The model under review builds one solid part; all positions refer to its coordinate system, in mm. A direction names the side the tool comes from. Give positions to 0.01 mm unless a question says otherwise; leave off trailing zeros. Write each loop counter-clockwise with the first axis right and the second up, starting at its lowest first coordinate (ties: lowest second). Pieces come first, ordered by that corner, then holes. Notation, with made-up numbers: (52.5, -39) - (93.5, -39) arc R21 ccw to (93.5, -8) - close; hole circle Ø4 at (36.25, 31). An arc over 180 degrees is marked (long way). Write item = value, one per line.
```python
from build123d import *

# Parameters (mm, degrees)
SKETCH_1_R               = 5
EXTRUDE_1_DEPTH          = 10
SKETCH_2_R               = 2
EXTRUDE_2_DEPTH          = 6
SKETCH_3_W               = 0.3
SKETCH_3_H               = 0.5
HOLE_WIZARD_M4_1_D       = 3.3
HOLE_WIZARD_M4_1_DEPTH   = 10.1
HOLE_WIZARD_M4_1_TIP     = 0.991420021
CHAMFER_1_SIZE           = 0.5
CUT_EXTRUDE_1_DEPTH      = 18.492855685
CUT_EXTRUDE_1_DEPTH_BACK = 18.492855685
SKETCH_6_R               = 2.25


with BuildPart() as part:
    # 草图1 → 凸台-拉伸1 (new, symmetric)
    with BuildSketch(Plane(origin=(0, 0, 0), x_dir=(1, 0, 0), z_dir=(0, 1, 0))):
        with Locations(Location((0, 0, 0), (0, 0, 270))):
            Circle(SKETCH_1_R)
    extrude(amount=EXTRUDE_1_DEPTH, both=True)

    # 草图2 → 凸台-拉伸2 (add)
    with BuildSketch(Plane.XZ.offset(10)):
        with Locations(Location((0, 0, 0), (0, 0, 90))):
            Circle(SKETCH_2_R)
    extrude(amount=EXTRUDE_2_DEPTH)

    # 草图3 → 切除-旋转1 (revolve, cut)
    with BuildSketch(Plane.XY, mode=Mode.PRIVATE) as cut_revolve_1_sk:
        with Locations((1.85, -10.25)):
            Rectangle(SKETCH_3_W, SKETCH_3_H)
    revolve(cut_revolve_1_sk.sketch.rotate(Axis((0, 0, 0), (0, -1, 0)), 90), axis=Axis((0, 0, 0), (0, -1, 0)), mode=Mode.SUBTRACT)

    # M4 螺纹孔1
    with Locations(Plane(origin=(0, 10, 0), x_dir=(1, 0, 0), z_dir=(0, 1, 0))):
        with Locations((0, 0)):
            Hole(HOLE_WIZARD_M4_1_D / 2, depth=HOLE_WIZARD_M4_1_DEPTH)
            with Locations((0, 0, -(HOLE_WIZARD_M4_1_DEPTH + HOLE_WIZARD_M4_1_TIP / 2))):  # 118° drill point
                Cone(0, HOLE_WIZARD_M4_1_D / 2, HOLE_WIZARD_M4_1_TIP, mode=Mode.SUBTRACT)

    # 倒角1
    chamfer_1_edges = [part.edges().sort_by_distance(p)[0] for p in [
        (0, -10, -5),
        (0, 10, -5),
    ]]
    chamfer(chamfer_1_edges, length=CHAMFER_1_SIZE)

    # 草图6 → 切除-拉伸1 (cut, two sides: drawn at the far end of the back side and taken through both)
    with BuildSketch(Plane(origin=(0, 0, 0), x_dir=(0, 0, -1), z_dir=(1, 0, 0)).offset(-CUT_EXTRUDE_1_DEPTH_BACK)):
        Circle(SKETCH_6_R)
    extrude(amount=CUT_EXTRUDE_1_DEPTH + CUT_EXTRUDE_1_DEPTH_BACK, mode=Mode.SUBTRACT)


solid = part.part
```
1. Machinability: for faces 4 (the flat face through (-2, 10, 0)), 5 (the cylindrical face through (1.66, -10.25, -0.37)), 6 (the cylindrical face through (2, -13, 0)), which of the approach directions +Z, -Z, +X, -X, +Y, -Y give a long, thin tool a straight path to every point of the face, cutting with its end or side? Answer none if there is none.
Findings below:
face_4 = +Z, -Z, +X, -X, +Y
face_5 = none
face_6 = -Y
2. For line 1 (Y direction, x = 3.25, z = 0); line 2 (Z direction, x = 0.25, y = 0); line 3 (Y direction, x = -1.75, z = 0.25), list the stretches that pass through material, from the lowest coordinate up. Write a range as from..to.
Findings below:
line_1 = -10..-2.25, 2.25..10
line_2 = -4.99..-2.25, 2.25..4.99
line_3 = -16..-10.5, -10..-2.24, 2.24..10
3. Insertion check: P1, Ø6, axis at y = 0, z = 0, coming from the +X side; P2, Ø3, axis at y = -8.5, z = -2, coming from the -X side; P3, Ø1, axis at x = 1, z = -0.5, coming from the +Y side; P4, Ø4, axis at x = 3.5, y = 5, coming from the +Z side. Each pin has a flat end and moves straight along its axis. Give the tip position at first contact, or say it passes through.
Findings below:
P1 = 5
P2 = -4.97
P3 = -2.02
P4 = 4.77
4. Take a section at B-B on x = 0. Give the boundary of the cut face in (y, z).
Findings below:
outline = (-16, -2) - (-10.5, -2) - (-10.5, -1.7) - (-10, -1.7) - (-10, -4.5) - (-9.5, -5) - (9.5, -5) - (10, -4.5) - (10, -1.65) - (1.53, -1.65) arc R2.25 cw (long way) to (1.53, 1.65) - (10, 1.65) - (10, 4.5) - (9.5, 5) - (-9.5, 5) - (-10, 4.5) - (-10, 1.7) - (-10.5, 1.7) - (-10.5, 2) - (-16, 2) - close
5. Take a section at A-A on z = 0. Give the boundary of the cut face in (x, y), and give its area (3 significant figures).
Findings below:
outline = (-5, -9.5) - (-4.5, -10) - (-1.7, -10) - (-1.7, -10.5) - (-2, -10.5) - (-2, -16) - (2, -16) - (2, -10.5) - (1.7, -10.5) - (1.7, -10) - (4.5, -10) - (5, -9.5) - (5, -2.25) - (-5, -2.25) - close; (-5, 2.25) - (-1.65, 2.25) - (-1.65, 10) - (-4.5, 10) - (-5, 9.5) - close; (1.65, 2.25) - (5, 2.25) - (5, 9.5) - (4.5, 10) - (1.65, 10) - close
area = 153 mm²
6. Take a section at D-D on y = 1.25. Give the boundary of the cut face in (x, z), and give its area (3 significant figures).
Findings below:
outline = (-4.64, -1.87) arc R5 ccw to (4.64, -1.87) - close; (-4.64, 1.87) - (4.64, 1.87) arc R5 ccw to start
area = 42.0 mm²
7. Take a section at C-C on y = 6. Give the boundary of the cut face in (x, z).
Findings below:
outline = circle Ø10 at (0, 0); hole circle Ø3.3 at (0, 0)
8. Draft analysis for pull direction X (two halves, no side actions). For faces 1 (the cylindrical face through (-1.524, 5.706, 0.632)), 2 (the flat face through (0, -16, 0)), 3 (the cylindrical face through (-1.915, 0.133, 4.619)), state which applies: +X half, -X half, draft (parallel to the pull), parting line (faces both ways), or undercut.
Findings below:
face_1 = undercut
face_2 = draft
face_3 = parting line
